The drawing under review shows one solid part. Ordinate dimensions are in mm from its lowest x, y, z. Round coordinates to 2 decimals unless told otherwise and drop trailing zeros. Order: outer loops, then holes, each group sorted by start corner. A loop starts at its lowest first (then second) coordinate and runs counter-clockwise, first axis right, second up. Notation, with made-up numbers: M 87,-40 L 127,-40 A35 ccw 127,-1 Z; hole C 6.25,10.25 d7. An arc over 180 degrees is marked long. Answer as a JSON object with one key per item and string values.
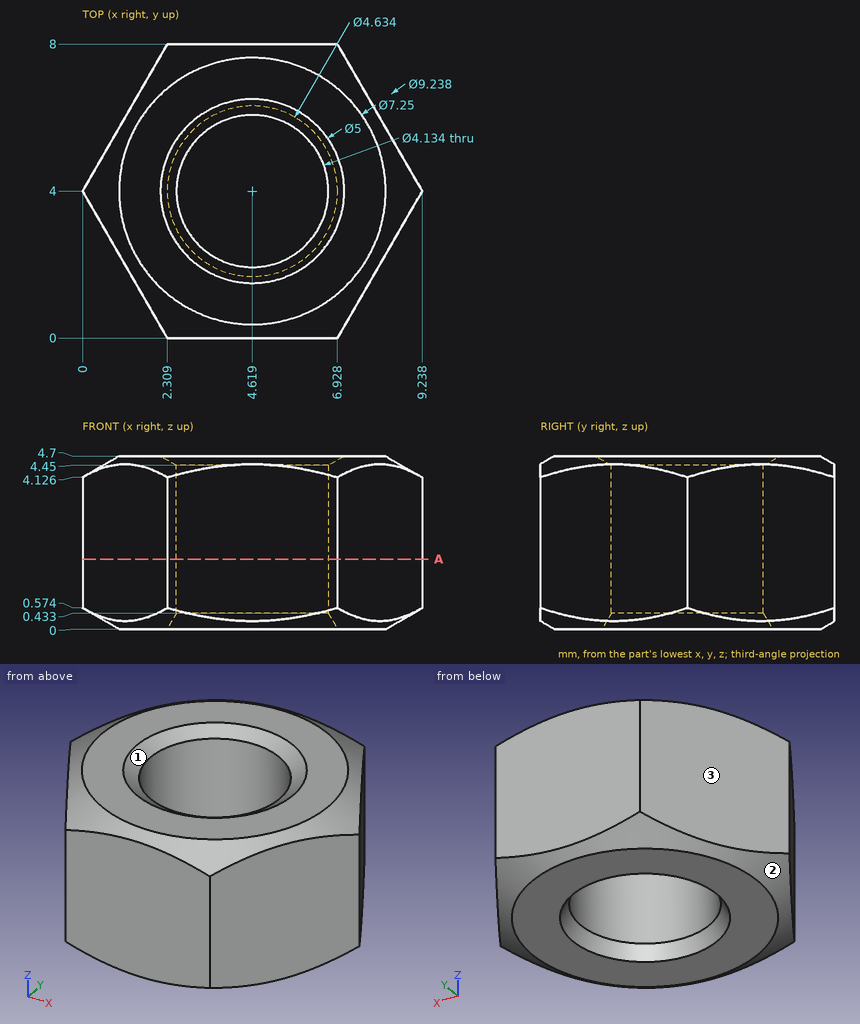
1) Mouldability with a two-part tool opening along Y and no side actions: class the marked faces 1, 2 and 3 as +Y half, -Y half, draft (parallel to the pull), parting line (faces both ways), or undercut.
Geometry check:
{"face 1": "undercut", "face 2": "parting line", "face 3": "+Y half"}
2) Add section A-A on z = 1.9. State the section outline as (x, y) points (1 decimal), and give its area (3 significant figures).
Geometry check:
{"outline": "M 0,4 L 2.3,0 L 6.9,0 L 9.2,4 L 6.9,8 L 2.3,8 Z; hole C 4.6,4 d4.1", "area": "42.0 mm²"}
3) Insertion check: P1, Ø1, axis at y = 2.5, z = 2.5, coming from the +X side; P2, Ø1, axis at x = 7, z = 2.5, coming from the -Y side; P3, Ø2, axis at y = 1, z = 1, coming from the -X side (1 decimal). Each pin has a flat end and moves straight along its axis. Give the tip position at first contact, or say it passes through.
Geometry check:
{"P1": "stops at x = 8.66", "P2": "stops at y = 0", "P3": "stops at x = 1.2"}
4) For L1, parallel to X at y = 2.75, z = 3.6 (1 decimal); L2, parallel to Y at x = 5.5, z = 1.75; L3, parallel to X at y = 5.5, z = 1.15 (1 decimal), list the stretches that pass through material, from the lowest coordinate up.
Geometry check:
{"L1": "x = 0.7 to 3, 6.3 to 8.5", "L2": "y = 0 to 2.13, 5.87 to 8", "L3": "x = 0.9 to 3.2, 6 to 8.4"}
